Geometry: see drawing. Coordinates: mm, zero at the bounding-box minimum. A direction names the side the tool comes from. Coordinates: 2 decimals unless noted, no trailing zeros. Write each loop counter-clockwise with the first axis right and the second up, starting at its lowest first coordinate (ties: lowest second). Pieces come first, ordered by that corner, then holes. Notation, with made-up numbers: (52, 38) - (56, 38) arc R17 ccw to (56, 50) - close; hole circle Ø1 at (39, 18.25). An arc over 180 degrees is marked (long way). One line per question, with ' | ' between items. Start each with the question number.
1) Section query D-D on x = 112. Return loops of the section in (y, z) (1 decimal).
2) Section query A-A on x = 35. Return loops of the section in (y, z).
3) Draft query along Y for the marked faces 1, 2 and 3. Return one class per face: released by +Y, released by -Y, zero draft, split by the parting line, or undercut.
4) Reachability of the marked faces 4, 5 and 6 from +Z, -Z, +X, -X, +Y, -Y: full face, straight path, thin tool, end or side. Return the list, or none.
5) Section query C-C on y = 36.5. Return loops of the section in (x, z).
6) First-contact query: P1, Ø6, axis at x = 127, y = 43.5, coming from the +Z side; P2, Ø22, axis at y = 82.5, z = 55.5, coming from the +X side; P3, Ø12, axis at x = 20.5, y = 92, coming from the -Z side. Flat tips, straight axial feed; report the tip coordinate or a pass-through.
7) Section query B-B on z = 21. Return loops of the section in (x, y), and give its area (3 significant figures).
8) Line query: line 1 (Y direction, x = 136, z = 100.5); line 2 (X direction, y = 86, z = 35); line 3 (Z direction, x = 99, y = 42.5). Output: solid intervals per line, ascending.
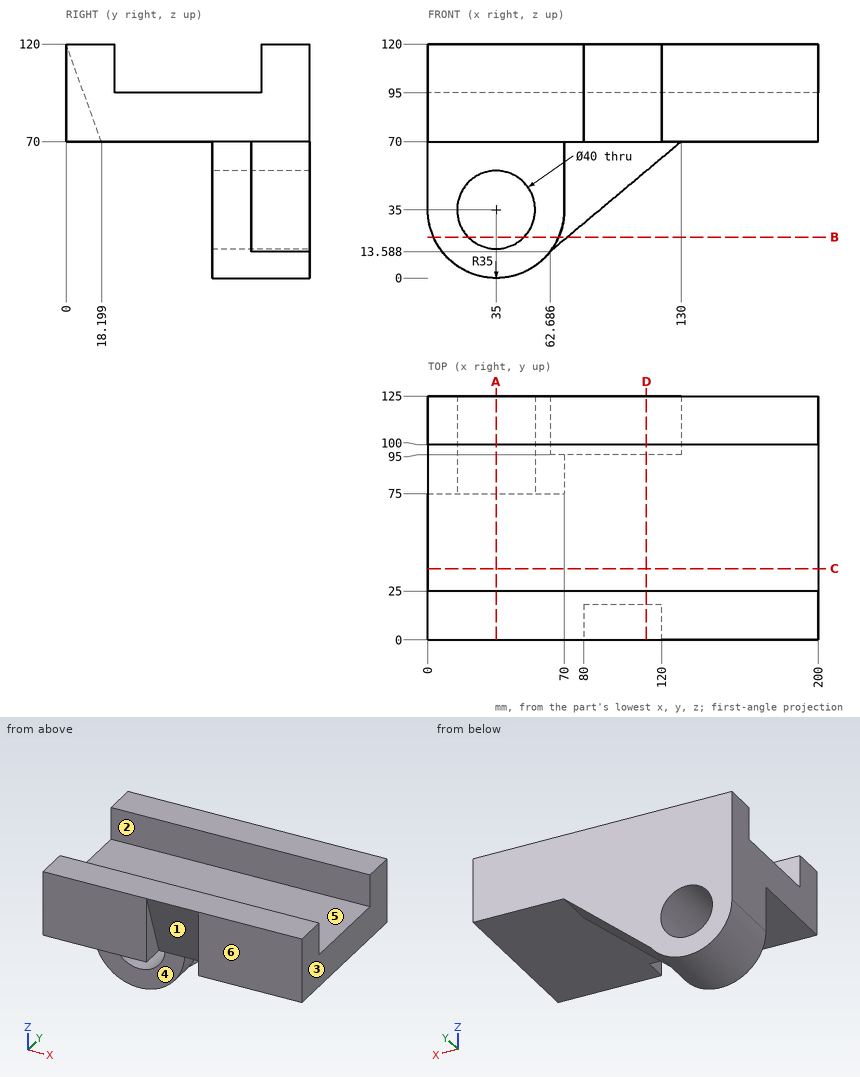
Answer key:
1) outline: (0, 120) - (18.2, 70) - (95, 70) - (95, 54.9) - (125, 54.9) - (125, 120) - (100, 120) - (100, 95) - (25, 95) - (25, 120) - close
2) outline: (0, 70) - (75, 70) - (75, 55) - (125, 55) - (125, 120) - (100, 120) - (100, 95) - (25, 95) - (25, 120) - (0, 120) - close; (75, 0) - (125, 0) - (125, 15) - (75, 15) - close
3) face 1: released by -Y | face 2: undercut | face 3: zero draft
4) face 4: -Z, +X, -X, -Y | face 5: +Z, +X, -X | face 6: +Z, -Z, +X, -X, -Y
5) outline: (0, 70) - (200, 70) - (200, 95) - (0, 95) - close
6) P1: z = 95 | P2: x = 70 | P3: z = 1.05
7) outline: (2.92, 75) - (20.72, 75) - (20.72, 125) - (2.92, 125) - close; (49.28, 75) - (67.08, 75) - (67.08, 95) - (71.53, 95) - (71.53, 125) - (49.28, 125) - close | area: 1,910 mm²
8) line 1: 0 to 25, 100 to 125 | line 2: 0 to 15, 55 to 70 | line 3: 70 to 95
